Source: CAD feature listing. Evaluate the final solid. Frame: model axes, mm. A direction names the side the tool comes from. Give positions to 0.01 mm unless a question says otherwise; leave off trailing zeros. Order: outer loops, then holes, each group sorted by start corner. A loop starts at its lowest first (then second) coordinate and runs counter-clockwise, first axis right, second up.
1) Material intervals for line 1 (Y direction, x = 0, z = -4.75); line 2 (X direction, y = 3.75, z = -7), sorted ascending.
2) Access query for faces 1 (the face through (-1, 5, 13)), 2 (the face through (5, 0, 10)), 3 (the face through (1, -3, 0)), 4 (the face through (0.25, -6, -13)), 5 (the face through (5, -5, -5)). Directions: +Z, -Z, +X, -X, +Y, -Y. A direction counts if a zero-diameter tool reaches every point of the face in a straight line with its end or side. Return the directions, or none.
3) Section A-A, the plane z = -8.5. Give the number of separate pieces and of enclosed holes in the cut face, plus the area to 3 significant figures.
4) Section B-B, the plane z = 1.5. Return loops of the section in (x, y), plus the area to 3 significant figures.
5) Draft query along X for faces 6 (the face through (-5.54, 2.3, 7.4)), 7 (the face through (2.821, -6.911, -17.535)), 8 (the face through (3, 3, 15)), 9 (the face through (-0.25, 6, -13)). Return one class per face: released by +X, released by -X, zero draft, split by the parting line, or undercut.
6) First-contact query: P1, Ø6, axis at x = -4.5, z = -12.5, coming from the -Y side; P2, Ø7.5, axis at x = -7.5, z = -11.5, coming from the -Y side; P3, Ø0.6, axis at y = -4.5, z = 11.5, coming from the -X side; P4, Ø2.5, axis at x = 1, y = 1, coming from the +Z side. Flat tips, straight axial feed; report the tip coordinate or a pass-through.
```python
from build123d import *

# Parameters (mm, degrees)
SKETCH1_W          = 2
SKETCH1_H          = 15
CUT_EXTRUDE1_DEPTH = 15
CHAMFER1_SIZE      = 2
CUT_EXTRUDE2_DEPTH = 5


with BuildPart() as part:
    # Sketch1 → Revolve1 (revolve)
    with BuildSketch(Plane(origin=(0, 0, 0), x_dir=(1, 0, 0), z_dir=(0, 1, 0)), mode=Mode.PRIVATE) as revolve1_sk:
        Polygon((3, 20), (3, 0), (4, 0), (6, 0), (10, 0), (10, 15), (5, 20), align=None)
        with Locations((5, -7.5)):
            Rectangle(SKETCH1_W, SKETCH1_H)
    revolve(revolve1_sk.sketch.rotate(Axis((0, 0, -20), (0, 0, 1)), 180), axis=Axis((0, 0, -20), (0, 0, 1)))

    # Sketch2 → Cut-Extrude1 (cut)
    with BuildSketch(Plane(origin=(0, 0, -20), x_dir=(-1, 0, 0), z_dir=(0, 0, -1))):
        with BuildLine():
            ThreePointArc((-9.996874512, 0.25), (-10, 0), (-9.996874512, -0.25))
            Line((-9.996874512, -0.25), (-0.603553391, -0.25))
            Line((-0.603553391, -0.25), (-0.353553391, 0))
            Line((-0.353553391, 0), (-0.603553391, 0.25))
            Line((-0.603553391, 0.25), (-9.996874512, 0.25))
        make_face()
        with BuildLine():
            Line((-0.25, -0.25), (-0.603553391, -0.25))
            Line((-0.603553391, -0.25), (-7.245634453, -6.892081063))
            ThreePointArc((-7.245634453, -6.892081063), (-7.071067812, -7.071067812), (-6.892081063, -7.245634453))
            Line((-6.892081063, -7.245634453), (-0.25, -0.603553391))
            Line((-0.25, -0.603553391), (-0.25, -0.25))
        make_face()
        with BuildLine():
            Line((-7.245634453, 6.892081063), (-0.603553391, 0.25))
            Line((-0.603553391, 0.25), (-0.25, 0.25))
            Line((-0.25, 0.25), (-0.25, 0.603553391))
            Line((-0.25, 0.603553391), (-6.892081063, 7.245634453))
            ThreePointArc((-6.892081063, 7.245634453), (-7.071067812, 7.071067812), (-7.245634453, 6.892081063))
        make_face()
        with BuildLine():
            Line((0, -0.353553391), (-0.25, -0.603553391))
            Line((-0.25, -0.603553391), (-0.25, -9.996874512))
            ThreePointArc((-0.25, -9.996874512), (0, -10), (0.25, -9.996874512))
            Line((0.25, -9.996874512), (0.25, -0.603553391))
            Line((0.25, -0.603553391), (0, -0.353553391))
        make_face()
        with BuildLine():
            Line((-0.25, 9.996874512), (-0.25, 0.603553391))
            Line((-0.25, 0.603553391), (0, 0.353553391))
            Line((0, 0.353553391), (0.25, 0.603553391))
            Line((0.25, 0.603553391), (0.25, 9.996874512))
            ThreePointArc((0.25, 9.996874512), (0, 10), (-0.25, 9.996874512))
        make_face()
        with BuildLine():
            Line((0.603553391, -0.25), (0.25, -0.25))
            Line((0.25, -0.25), (0.25, -0.603553391))
            Line((0.25, -0.603553391), (6.892081063, -7.245634453))
            ThreePointArc((6.892081063, -7.245634453), (7.071067812, -7.071067812), (7.245634453, -6.892081063))
            Line((7.245634453, -6.892081063), (0.603553391, -0.25))
        make_face()
        with BuildLine():
            Line((0.353553391, 0), (0.603553391, -0.25))
            Line((0.603553391, -0.25), (9.996874512, -0.25))
            ThreePointArc((9.996874512, -0.25), (10, 0), (9.996874512, 0.25))
            Line((9.996874512, 0.25), (0.603553391, 0.25))
            Line((0.603553391, 0.25), (0.353553391, 0))
        make_face()
        with BuildLine():
            Line((0.25, 0.603553391), (0.25, 0.25))
            Line((0.25, 0.25), (0.603553391, 0.25))
            Line((0.603553391, 0.25), (7.245634453, 6.892081063))
            ThreePointArc((7.245634453, 6.892081063), (7.071067812, 7.071067812), (6.892081063, 7.245634453))
            Line((6.892081063, 7.245634453), (0.25, 0.603553391))
        make_face()
    extrude(amount=-CUT_EXTRUDE1_DEPTH, mode=Mode.SUBTRACT)

    # Chamfer1
    chamfer1_edges = [part.edges().sort_by_distance(p)[0] for p in [
        (10, 0, 0),
    ]]
    chamfer(chamfer1_edges, length=CHAMFER1_SIZE)

    # Sketch3 → Cut-Extrude2 (cut)
    with BuildSketch(Plane.XY.offset(15)):
        with BuildLine():
            Line((1, 3.872983346), (1, 5.916079783))
            ThreePointArc((1, 5.916079783), (0, 6), (-1, 5.916079783))
            Line((-1, 5.916079783), (-1, 3.872983346))
            ThreePointArc((-1, 3.872983346), (0, 4), (1, 3.872983346))
        make_face()
        with BuildLine():
            ThreePointArc((6, 0), (5.978983137, 0.501757562), (5.916079783, 1))
            Line((5.916079783, 1), (3.872983346, 1))
            ThreePointArc((3.872983346, 1), (3.968118785, 0.50401717), (4, 0))
            ThreePointArc((4, 0), (3.968118785, -0.50401717), (3.872983346, -1))
            Line((3.872983346, -1), (5.916079783, -1))
            ThreePointArc((5.916079783, -1), (5.978983137, -0.501757562), (6, 0))
        make_face()
        with BuildLine():
            ThreePointArc((-1, -5.916079783), (0, -6), (1, -5.916079783))
            Line((1, -5.916079783), (1, -3.872983346))
            ThreePointArc((1, -3.872983346), (0, -4), (-1, -3.872983346))
            Line((-1, -3.872983346), (-1, -5.916079783))
        make_face()
        with BuildLine():
            Line((-3.872983346, 1), (-5.916079783, 1))
            ThreePointArc((-5.916079783, 1), (-6, 0), (-5.916079783, -1))
            Line((-5.916079783, -1), (-3.872983346, -1))
            ThreePointArc((-3.872983346, -1), (-4, 0), (-3.872983346, 1))
        make_face()
    extrude(amount=-CUT_EXTRUDE2_DEPTH, mode=Mode.SUBTRACT)


solid = part.part
```
From the geometry:
1. line 1: y = -10 to -3, 3 to 10
1. line 2: x = -9.27 to -4.1, -3.4 to -0.25, 0.25 to 3.4, 4.1 to 9.27
2. face 1: +Z, +Y, -Y
2. face 2: +Z, +X, -X
2. face 3: +Z
2. face 4: -Z, +Y, -Y
2. face 5: -Z
3. separate pieces: 8
3. enclosed holes: 0
3. area: 258 mm2
4. outline: circle Ø12 at (0, 0); hole circle Ø8 at (0, 0)
4. area: 62.8 mm2
5. face 6: split by the parting line
5. face 7: released by +X
5. face 8: zero draft
5. face 9: undercut
6. P1: stops at y = -9.89
6. P2: stops at y = -9.27
6. P3: stops at x = -4.28
6. P4: passes through
